Design review of the part shown in the three views and the two pictorial views. Dimensions are in mm from the part's minimum x, y and z. A direction names the side the tool comes from. Give positions to 0.01 mm unless a question says otherwise; leave off trailing zeros. Loops run counter-clockwise (first coordinate to the right, second up) from the corner with the lowest first, then second, coordinate; pieces in that order, holes last. Notation, with made-up numbers: (69.25, 86.25) - (98.25, 86.25) arc R37 ccw to (98.25, 125.25) - close; hole circle Ø3 at (64.25, 87). An arc over 180 degrees is marked (long way). Answer in a Markdown table with one row per item.
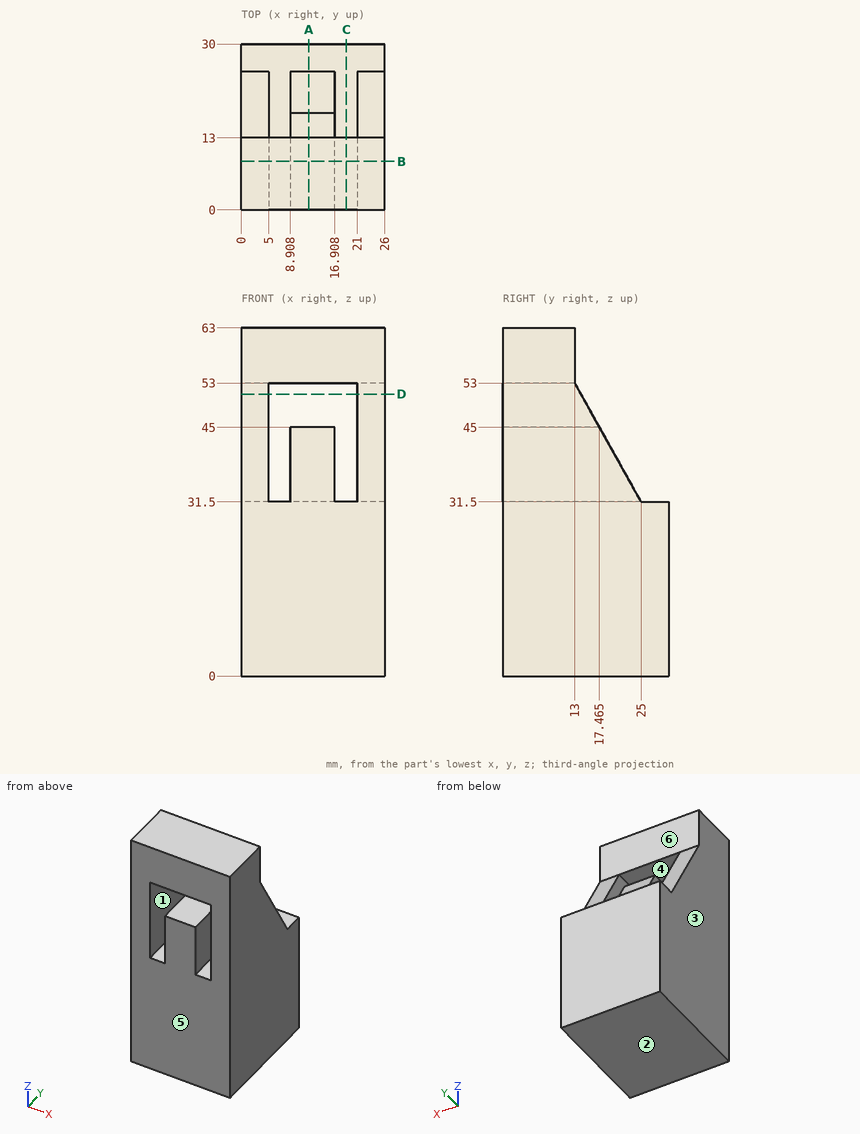
1. Wall thickness on line 1 (X direction, y = 15.25, z = 34); line 2 (X direction, y = 12.5, z = 47); line 3 (Z direction, x = 17.5, y = 3): over which ranges is each line inside the solid? List them lowest first. Write a range as [from, to].
Values:
| item | result |
|---|---|
| line 1 | x = [0, 5], [8.91, 16.91], [21, 26] |
| line 2 | x = [0, 5], [21, 26] |
| line 3 | z = [0, 31.5], [53, 63] |
2. Clearance check with flat-ended pins moving along their axes: pin 1 (8 mm diameter, centred on x = 14, z = 57, fed in from +Y); pin 2 (5 mm diameter, centred on x = 12.5, y = 23.5, fed in from +Z) (1 decimal); pin 3 (2 mm diameter, centred on x = 3, z = 41, fed in from +Y) (1 decimal). State where each tip first meets the part, or that it passes through.
Values:
| item | result |
|---|---|
| pin 1 | stops at y = 13 |
| pin 2 | stops at z = 38.7 |
| pin 3 | stops at y = 20.3 |
3. We need section A-A, the plane x = 12.25. Give the boundary of the cut face in (y, z) (1 decimal), and give its area (3 significant figures).
Values:
| item | result |
|---|---|
| outline | (0, 0) - (30, 0) - (30, 31.5) - (25, 31.5) - (17.5, 45) - (0, 45) - close; (0, 53) - (13, 53) - (13, 63) - (0, 63) - close |
| area | 1,360 mm^2 |
4. For the marked faces 4, 5 and 6, list the 3-axis set-ups (+Z, -Z, +X, -X, +Y, -Y) from which the entire face can be reached by the end or side of a thin tool; tool diameter is ignored.
Values:
| item | result |
|---|---|
| face 4 | +Y, -Y |
| face 5 | +Z, -Z, +X, -X, -Y |
| face 6 | +Z, +X, -X, +Y |
5. We need section C-C, the plane x = 19. Give the boundary of the cut face in (y, z).
Values:
| item | result |
|---|---|
| outline | (0, 0) - (30, 0) - (30, 31.5) - (0, 31.5) - close; (0, 53) - (13, 53) - (13, 63) - (0, 63) - close |
6. Mouldability with a two-part tool opening along X and no side actions: class the marked faces 1, 2 and 3 as released by +X, released by -X, zero draft, split by the parting line, or undercut.
Values:
| item | result |
|---|---|
| face 1 | undercut |
| face 2 | zero draft |
| face 3 | released by -X |
7. We need section D-D, the plane z = 51. Give the boundary of the cut face in (x, y), and give its area (3 significant figures).
Values:
| item | result |
|---|---|
| outline | (0, 0) - (5, 0) - (5, 14.12) - (0, 14.12) - close; (21, 0) - (26, 0) - (26, 14.12) - (21, 14.12) - close |
| area | 141 mm^2 |
8. We need section B-B, the plane y = 8.75. Give the boundary of the cut face in (x, z), and give its area (3 significant figures).
Values:
| item | result |
|---|---|
| outline | (0, 0) - (26, 0) - (26, 63) - (0, 63) - close; hole (5, 31.5) - (8.91, 31.5) - (8.91, 45) - (16.91, 45) - (16.91, 31.5) - (21, 31.5) - (21, 53) - (5, 53) - close |
| area | 1,400 mm^2 |
